Design review of the part built by this model. Coordinates are the model's own, in mm. Coordinates: 2 decimals unless noted, no trailing zeros. Write each loop counter-clockwise with the first axis right and the second up, starting at its lowest first coordinate (ties: lowest second). Pieces come first, ordered by that corner, then holes. Notation, with made-up numbers: M 72,21 L 131,21 A22 ccw 131,44 Z; hole C -38.5,-16 d8. An arc over 180 degrees is marked long. One line per question, with ' | ' between items.
from build123d import *

# Parameters (mm, degrees)
SKETCH1_W      = 101.6
SKETCH1_H      = 203.2
EXTRUDE1_DEPTH = 7
CHAMFER1_SIZE  = 25


with BuildPart() as part:
    # Sketch1 → Extrude1 (new, symmetric)
    with BuildSketch(Plane.XY):
        with Locations((50.8, 101.6)):
            Rectangle(SKETCH1_W, SKETCH1_H)
    extrude(amount=EXTRUDE1_DEPTH, both=True)

    # Chamfer1
    chamfer1_edges = [part.edges().sort_by_distance(p)[0] for p in [
        (0, 203.2, 0),
    ]]
    chamfer(chamfer1_edges, length=CHAMFER1_SIZE)


solid = part.part
1. To check wall thickness, follow line 1 along X through (y, z) = (181.5, 0.25); line 2 along Y through (x, z) = (23, 0.5); line 3 along Y through (x, z) = (7.5, 2). State the ranges of each line that lie inside material, in increasing order. Write a range as [from, to].
Answer sheet:
line 1: [3.3, 101.6] | line 2: [0, 201.2] | line 3: [0, 185.7]
2. Take a section at B-B (x = 13.5). Write out the cut boundary in (y, z), then the cut area to 3 significant figures.
Answer sheet:
outline: M 0,-7 L 191.7,-7 L 191.7,7 L 0,7 Z | area: 2,680 mm^2
3. Take a section at A-A (z = -0.5). Write out the cut boundary in (x, y), then the cut area to 3 significant figures.
Answer sheet:
outline: M 0,0 L 101.6,0 L 101.6,203.2 L 25,203.2 L 0,178.2 Z | area: 20,300 mm^2
